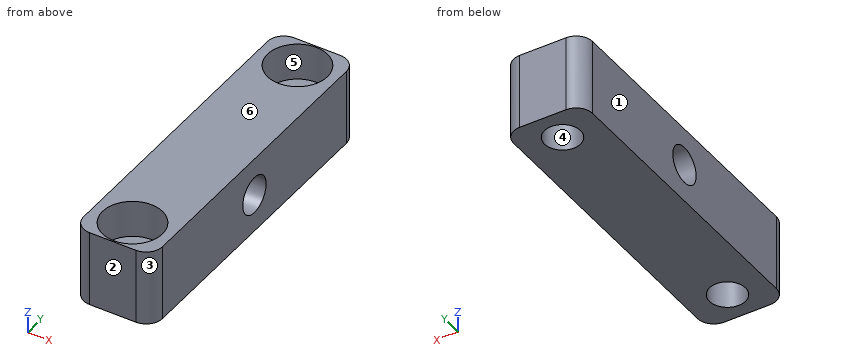
from build123d import *

# Parameters (mm, degrees)
SKETCH_1_W                = 14.5
SKETCH_1_H                = 59.5
EXTRUDE_1_DEPTH           = 14
FILLET_1_R                = 3
HOLE_WIZARD_2_D           = 6.6
HOLE_WIZARD_2_CBORE_D     = 11
HOLE_WIZARD_2_CBORE_DEPTH = 6.8
HOLE_WIZARD_M8_1_D        = 6.8


with BuildPart() as part:
    # 草图1 → 凸台-拉伸1 (new body)
    with BuildSketch(Plane.XY):
        Rectangle(SKETCH_1_W, SKETCH_1_H)
    extrude(amount=EXTRUDE_1_DEPTH)

    # 圆角1
    fillet_1_edges = [part.edges().sort_by_distance(p)[0] for p in [
        (7.25, -29.75, 7),
        (-7.25, -29.75, 7),
        (-7.25, 29.75, 7),
        (7.25, 29.75, 7),
    ]]
    fillet(fillet_1_edges, radius=FILLET_1_R)

    # 打孔尺寸(%根据)内六角圆柱头螺钉的类型2 (through all)
    with Locations(Plane.XY.offset(14)):
        with Locations((0, 24), (0, -24)):
            CounterBoreHole(HOLE_WIZARD_2_D / 2, HOLE_WIZARD_2_CBORE_D / 2, HOLE_WIZARD_2_CBORE_DEPTH)

    # M8 螺纹孔1 (through all)
    with Locations(Plane.ZY.offset(7.25)):
        with Locations((7, 0)):
            Hole(HOLE_WIZARD_M8_1_D / 2)


solid = part.part
Source: CAD feature listing. Evaluate the final solid. Frame: model axes, mm. Face numbers are marked on the shaded views. A direction names the side the tool comes from. Give positions to 0.01 mm unless a question says otherwise; leave off trailing zeros. Write each loop counter-clockwise with the first axis right and the second up, starting at its lowest first coordinate (ties: lowest second). Pieces come first, ordered by that corner, then holes. Notation, with made-up numbers: M 18,77.25 L 45,77.25 A9 cw 45,92.25 Z; hole C 37,76.25 d7. An arc over 180 degrees is marked long. Return JSON: item names as keys, results as strings. Group by question number.
1) Set-up query: the marked faces 5 and 6. Return all of +Z, -Z, +X, -X, +Y, -Y with unobstructed straight access to the full face (end or side cutting, diameter ignored); none if empty.
2) Cut plane D-D, the plane z = 2.75. Output: boundary loops of the cut face in (x, y).
3) Pull-direction query (X, two-part tool) for the marked faces 1, 2, 3 and 4; classes: pulls with the +X half, pulls with the -X half, needs draft (parallel to the pull), parting line crosses it, or undercut.
4) Cut plane A-A, the plane x = 0. Output: boundary loops of the cut face in (y, z), plus the area to 3 significant figures.
5) Cut plane B-B, the plane y = 24. Output: boundary loops of the cut face in (x, z), plus the area to 3 significant figures.
6) Cut plane C-C, the plane z = 9.75. Output: boundary loops of the cut face in (x, y), plus the area to 3 significant figures.
7) Material intervals for line 1 along Y through (x, z) = (0, 3); line 2 along Y through (x, z) = (0, 11.5); line 3 along Y through (x, z) = (0, 9), sorted ascending. Write a range as [from, to].
Recorded:
{
 "1": {"face 5": "+Z", "face 6": "+Z, +X, -X, +Y, -Y"},
 "2": {"outline": "M -7.25,-26.75 A3 ccw -4.25,-29.75 L 4.25,-29.75 A3 ccw 7.25,-26.75 L 7.25,26.75 A3 ccw 4.25,29.75 L -4.25,29.75 A3 ccw -7.25,26.75 Z; hole C 0,-24 d6.6; hole C 0,24 d6.6"},
 "3": {"face 1": "pulls with the -X half", "face 2": "needs draft", "face 3": "pulls with the +X half", "face 4": "undercut"},
 "4": {"outline": "M -29.75,0 L -27.3,0 L -27.3,7.2 L -29.5,7.2 L -29.5,14 L -29.75,14 Z; M -20.7,0 L 20.7,0 L 20.7,7.2 L 18.5,7.2 L 18.5,14 L -18.5,14 L -18.5,7.2 L -20.7,7.2 Z; M 27.3,0 L 29.75,0 L 29.75,14 L 29.5,14 L 29.5,7.2 L 27.3,7.2 Z; hole C 0,7 d6.8", "area": "552 mm²"},
 "5": {"outline": "M -7.25,0 L -3.3,0 L -3.3,7.2 L -5.5,7.2 L -5.5,14 L -7.25,14 Z; M 3.3,0 L 7.25,0 L 7.25,14 L 5.5,14 L 5.5,7.2 L 3.3,7.2 Z", "area": "80.7 mm²"},
 "6": {"outline": "M -7.25,-26.75 A3 ccw -4.25,-29.75 L 4.25,-29.75 A3 ccw 7.25,-26.75 L 7.25,-2 L -7.25,-2 Z; M -7.25,2 L 7.25,2 L 7.25,26.75 A3 ccw 4.25,29.75 L -4.25,29.75 A3 ccw -7.25,26.75 Z; hole C 0,-24 d11; hole C 0,24 d11", "area": "607 mm²"},
 "7": {"line 1": "y = [-29.75, -27.3], [-20.7, 20.7], [27.3, 29.75]", "line 2": "y = [-29.75, -29.5], [-18.5, 18.5], [29.5, 29.75]", "line 3": "y = [-29.75, -29.5], [-18.5, -2.75], [2.75, 18.5], [29.5, 29.75]"}
}
